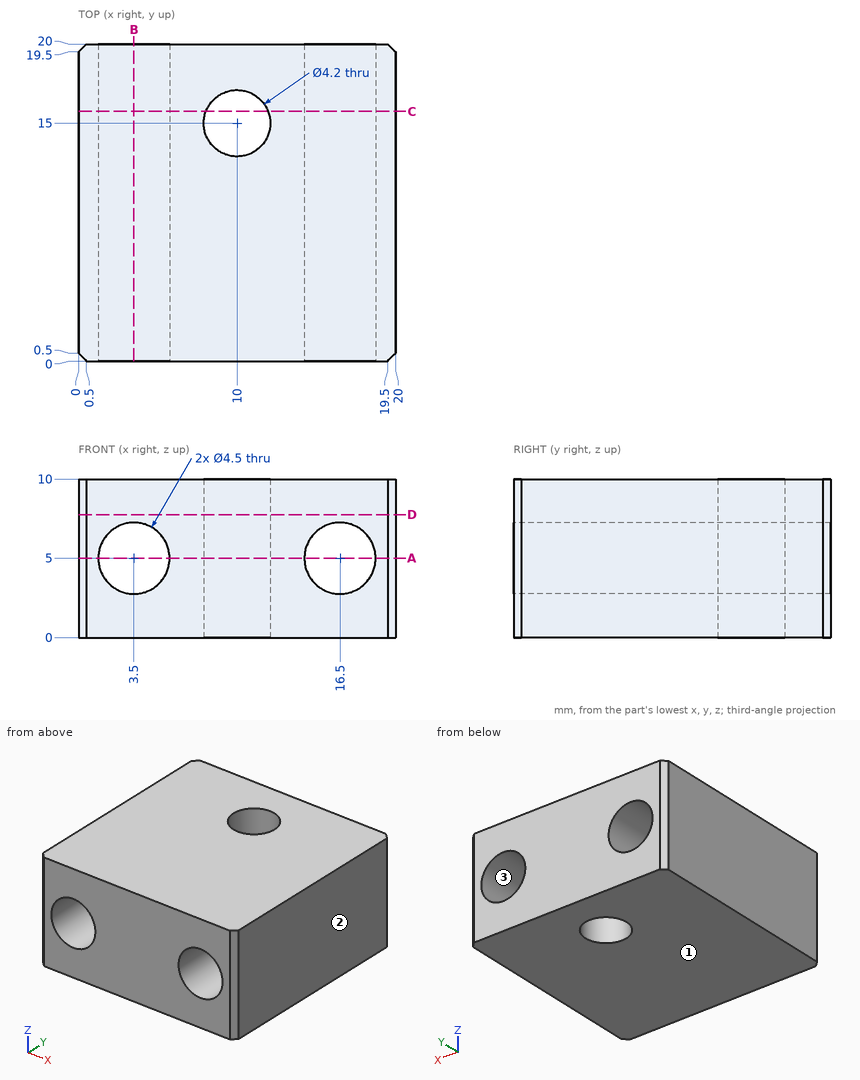
Can you work these out from the drawing? Everything is in mm from the part's minimum corner. Give positions to 0.01 mm unless a question says otherwise; leave off trailing zeros. Write each loop counter-clockwise with the first axis right and the second up, starting at its lowest first coordinate (ties: lowest second). Pieces come first, ordered by that corner, then holes. Notation, with made-up numbers: (9, 5.25) -> (68, 5.25) arc R23 cw to (68, 25.25) -> close; hole circle Ø10 at (14, -25.5). An arc over 180 degrees is marked (long way). Write each question's results on one line, items separated by ' | '.
Item 1: Suppose I cut it at A-A on z = 5. Write out the boundary of the cut face in (x, y).
Output:
outline: (0, 0.5) -> (0.5, 0) -> (1.25, 0) -> (1.25, 20) -> (0.5, 20) -> (0, 19.5) -> close; (5.75, 0) -> (14.25, 0) -> (14.25, 20) -> (5.75, 20) -> close; (18.75, 0) -> (19.5, 0) -> (20, 0.5) -> (20, 19.5) -> (19.5, 20) -> (18.75, 20) -> close; hole circle Ø4.2 at (10, 15)
Item 2: Suppose I cut it at D-D on z = 7.75. Write out the boundary of the cut face in (x, y), plus the area to 3 significant figures.
Output:
outline: (0, 0.5) -> (0.5, 0) -> (19.5, 0) -> (20, 0.5) -> (20, 19.5) -> (19.5, 20) -> (0.5, 20) -> (0, 19.5) -> close; hole circle Ø4.2 at (10, 15) | area: 386 mm^2
Item 3: Suppose I cut it at C-C on y = 15.75. Write out the boundary of the cut face in (x, z), plus the area to 3 significant figures.
Output:
outline: (0, 0) -> (8.04, 0) -> (8.04, 10) -> (0, 10) -> close; (11.96, 0) -> (20, 0) -> (20, 10) -> (11.96, 10) -> close; hole circle Ø4.5 at (3.5, 5); hole circle Ø4.5 at (16.5, 5) | area: 129 mm^2
Item 4: We'd pull the mould along X, two halves only. Please class the marked faces 1, 2 and 3: pulls with the +X half, pulls with the -X half, needs draft (parallel to the pull), parting line crosses it, or undercut.
Output:
face 1: needs draft | face 2: pulls with the +X half | face 3: undercut
Item 5: Suppose I cut it at B-B on x = 3.5. Write out the boundary of the cut face in (y, z).
Output:
outline: (0, 0) -> (20, 0) -> (20, 2.75) -> (0, 2.75) -> close; (0, 7.25) -> (20, 7.25) -> (20, 10) -> (0, 10) -> close
Item 6: For pin 1 Ø5 at (x, z) = (16.5, 5) entering from +Y; pin 2 Ø2.5 at (x, z) = (3.5, 5) entering from +Y, each with a flat end and sliding along its axis, tell me the tip position at first contact or that it passes through.
Output:
pin 1: stops at y = 20 | pin 2: passes through
Item 7: If I drill on L1, parallel to Z at x = 3.5, y = 9.75; L2, parallel to Y at x = 10, z = 7.25; L3, parallel to X at y = 5.75, z = 4.25, over which ranges is the centre line in solid material (lowest first)?
Output:
L1: z = 0 to 2.75, 7.25 to 10 | L2: y = 0 to 12.9, 17.1 to 20 | L3: x = 0 to 1.38, 5.62 to 14.38, 18.62 to 20
